The figure shows three views and two pictorial views of one solid part (mm, origin at its lowest corner). Answer the questions. Round coordinates to 2 decimals unless told otherwise and drop trailing zeros. Order: outer loops, then holes, each group sorted by start corner. A loop starts at its lowest first (then second) coordinate and runs counter-clockwise, first axis right, second up. Notation, with made-up numbers: (-40, 81) -> (-8, 81) arc R32 ccw to (-8, 113) -> close; hole circle Ø3 at (59, 51.25). An arc over 180 degrees is marked (long way). Answer as a JSON object with one key per item and string values. Group by question number.
Item 1: Given P1, Ø1, axis at x = 31.5, y = 2, coming from the -Z side; P2, Ø5, axis at y = 4.5, z = 195.5, coming from the +X side, each flat-ended and moving along its own axis, determine where each tip first touches the part or whether it passes through.
Item 2: Section C-C, the plane z = 159 is taken. Write down the section's boundary in (x, y), plus the area to 3 significant figures.
Item 3: Consider probe 1 along X at (y, z) = (4.5, 213); probe 2 along X at (y, z) = (9.5, 92); probe 3 along Z at (x, y) = (7, 7). Determine where each line is inside the solid, lowest interval first. Write a range as from..to.
Item 4: Section B-B, the plane x = 78.5 is taken. Write down the section's boundary in (y, z).
Item 5: Section A-A, the plane y = 8.5 is taken. Write down the section's boundary in (x, z).
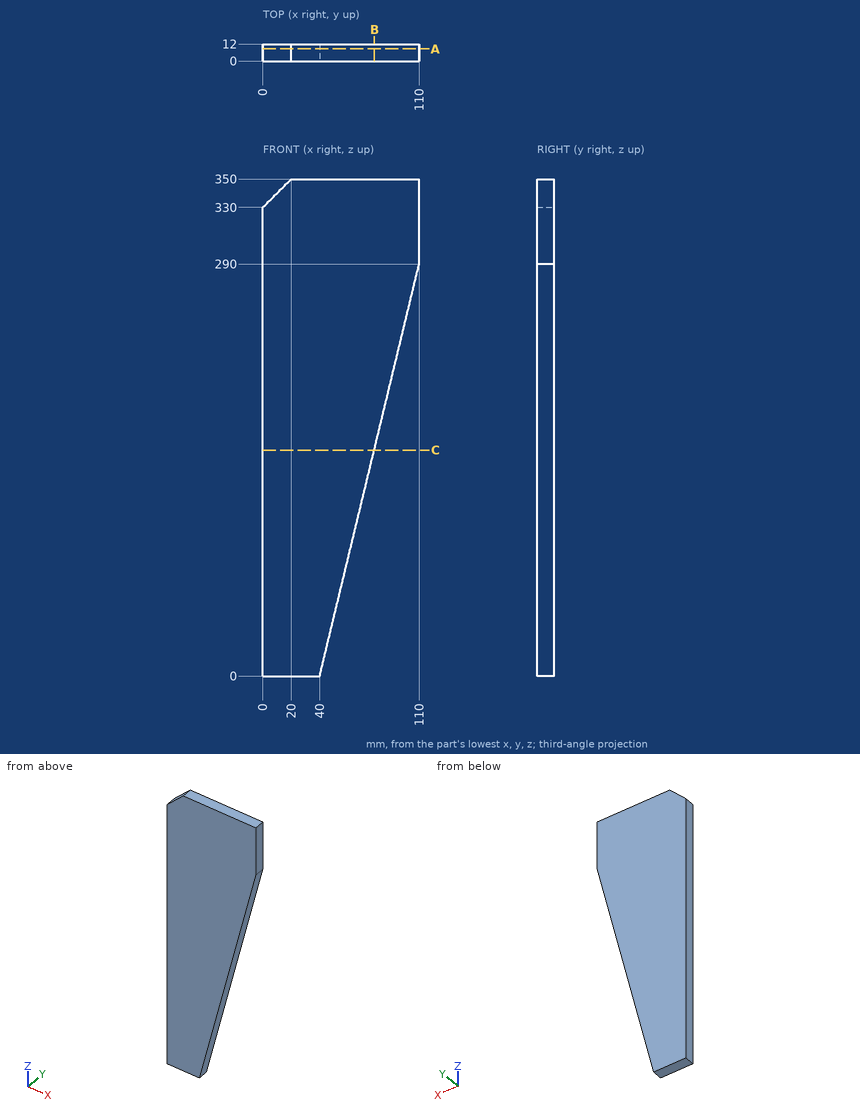
Values found:
{
 "1": {"P1": "z = 0", "P2": "x = 87.79"},
 "2": {"outline": "(0, 0) -> (78.38, 0) -> (78.38, 12) -> (0, 12) -> close", "area": "941 mm2"},
 "3": {"probe 1": "0..91.41", "probe 2": "0..62.21", "probe 3": "0..337"},
 "4": {"outline": "(0, 159.5) -> (12, 159.5) -> (12, 350) -> (0, 350) -> close"},
 "5": {"outline": "(0, 0) -> (40, 0) -> (110, 290) -> (110, 350) -> (20, 350) -> (0, 330) -> close"}
}
